```python
from build123d import *

# Parameters (mm, degrees)
SKETCH1_W              = 170
SKETCH1_H              = 100
BOSS_EXTRUDE1_DEPTH    = 15
M12_TAPPED_HOLE1_D     = 10.2
M12_TAPPED_HOLE1_DEPTH = 29.25
M12_TAPPED_HOLE1_TIP   = 3.064389157


with BuildPart() as part:
    # Sketch1 → Boss-Extrude1 (new body)
    with BuildSketch(Plane.XY):
        Rectangle(SKETCH1_W, SKETCH1_H)
    extrude(amount=BOSS_EXTRUDE1_DEPTH)

    # M12 Tapped Hole1
    with Locations(Plane.XY.offset(15)):
        with Locations((-55, 30), (0, 30), (55, 30), (55, -30), (0, -30), (-55, -30)):
            Hole(M12_TAPPED_HOLE1_D / 2, depth=M12_TAPPED_HOLE1_DEPTH)
            with Locations((0, 0, -(M12_TAPPED_HOLE1_DEPTH + M12_TAPPED_HOLE1_TIP / 2))):  # 118° drill point
                Cone(0, M12_TAPPED_HOLE1_D / 2, M12_TAPPED_HOLE1_TIP, mode=Mode.SUBTRACT)


solid = part.part
```
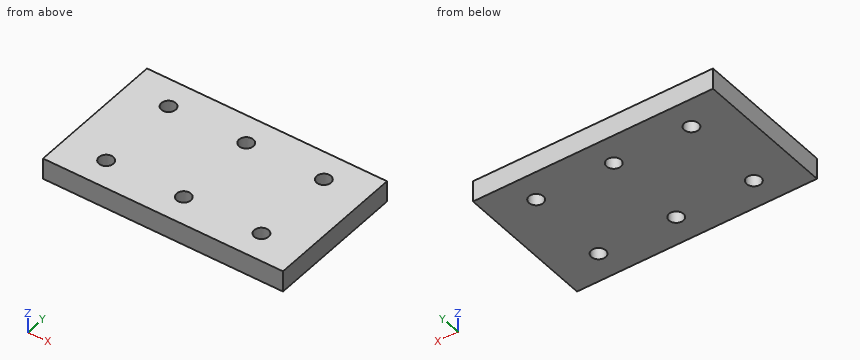
Build history of the part. All positions in model axes, mm. Give positions to 0.01 mm unless a question says otherwise; leave off trailing zeros. Loops run counter-clockwise (first coordinate to the right, second up) from the corner with the lowest first, then second, coordinate; pieces in that order, holes last.
1) Band-saw the part on C-C on z = 3.75. List the corners of the cut face in (x, y).
Values follow:
outline: (-85, -50) - (85, -50) - (85, 50) - (-85, 50) - close; hole circle Ø10.2 at (-55, -30); hole circle Ø10.2 at (-55, 30); hole circle Ø10.2 at (0, -30); hole circle Ø10.2 at (0, 30); hole circle Ø10.2 at (55, -30); hole circle Ø10.2 at (55, 30)
2) Probe line 1 along Y through (x, z) = (0, 3.25); line 2 along X through (y, z) = (33, 13.25); line 3 along Y through (x, z) = (-57, 10). List the from-to ranges inside material, lowest first.
Values follow:
line 1: y = -50 to -35.1, -24.9 to 24.9, 35.1 to 50
line 2: x = -85 to -59.12, -50.88 to -4.12, 4.12 to 50.88, 59.12 to 85
line 3: y = -50 to -34.69, -25.31 to 25.31, 34.69 to 50
3) Band-saw the part on A-A on y = -30. List the corners of the cut face in (x, z).
Values follow:
outline: (-85, 0) - (-60.1, 0) - (-60.1, 15) - (-85, 15) - close; (-49.9, 0) - (-5.1, 0) - (-5.1, 15) - (-49.9, 15) - close; (5.1, 0) - (49.9, 0) - (49.9, 15) - (5.1, 15) - close; (60.1, 0) - (85, 0) - (85, 15) - (60.1, 15) - close
4) Band-saw the part on B-B on x = 55. List the corners of the cut face in (y, z), then the cut area to 3 significant figures.
Values follow:
outline: (-50, 0) - (-35.1, 0) - (-35.1, 15) - (-50, 15) - close; (-24.9, 0) - (24.9, 0) - (24.9, 15) - (-24.9, 15) - close; (35.1, 0) - (50, 0) - (50, 15) - (35.1, 15) - close
area: 1,190 mm2
5) Band-saw the part on D-D on x = -53. List the corners of the cut face in (y, z).
Values follow:
outline: (-50, 0) - (-34.69, 0) - (-34.69, 15) - (-50, 15) - close; (-25.31, 0) - (25.31, 0) - (25.31, 15) - (-25.31, 15) - close; (34.69, 0) - (50, 0) - (50, 15) - (34.69, 15) - close
